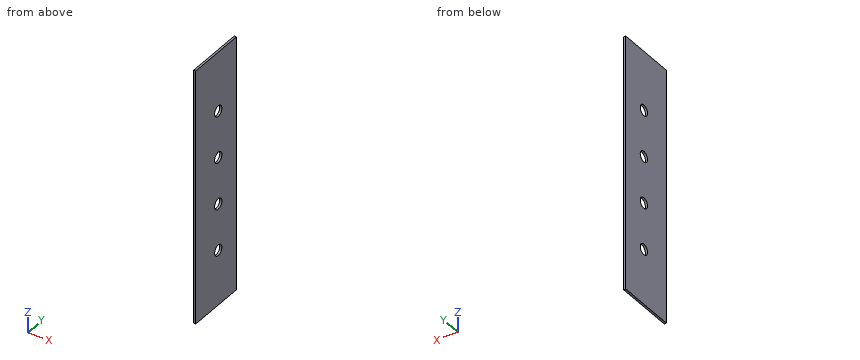
from build123d import *

# Parameters (mm, degrees)
SKETCH1_W           = 1200
SKETCH1_H           = 280
BOSS_EXTRUDE1_DEPTH = 10
SKETCH2_R           = 25
CUT_EXTRUDE1_DEPTH  = 10
LPATTERN1_COUNT     = 4
LPATTERN1_PITCH     = 220


with BuildPart() as part:
    # Sketch1 → Boss-Extrude1 (new body)
    with BuildSketch(Plane(origin=(0, 0, 0), x_dir=(0, 0, -1), z_dir=(1, 0, 0))):
        Rectangle(SKETCH1_W, SKETCH1_H)
    extrude(amount=BOSS_EXTRUDE1_DEPTH)

    # Sketch2 → Cut-Extrude1 (cut)
    with BuildSketch(Plane(origin=(10, 0, 0), x_dir=(0, 0, -1), z_dir=(1, 0, 0))):
        with Locations((-320, 15)):
            Circle(SKETCH2_R)
    cut_extrude1 = extrude(amount=-CUT_EXTRUDE1_DEPTH, mode=Mode.SUBTRACT)

    # LPattern1: Cut-Extrude1 ×4
    with Locations(*[(0, 0, -i * LPATTERN1_PITCH) for i in range(1, LPATTERN1_COUNT)]):
        add(cut_extrude1, mode=Mode.SUBTRACT)


solid = part.part
CAD build for the part. Positions are in the model's coordinates, mm. Round coordinates to 2 decimals unless told otherwise and drop trailing zeros. Write each loop counter-clockwise with the first axis right and the second up, starting at its lowest first coordinate (ties: lowest second). Pieces come first, ordered by that corner, then holes. Notation, with made-up numbers: (58, 20) -> (80, 20) arc R21 cw to (80, 37) -> close; hole circle Ø10 at (65.5, 49.25). An arc over 180 degrees is marked (long way). Answer as a JSON object with one key per item and string values.
(1) Band-saw the part on B-B, the plane x = 7.5. List the corners of the cut face in (y, z).
Reported:
{"outline": "(-140, -600) -> (140, -600) -> (140, 600) -> (-140, 600) -> close; hole circle Ø50 at (15, -340); hole circle Ø50 at (15, -120); hole circle Ø50 at (15, 100); hole circle Ø50 at (15, 320)"}
(2) Band-saw the part on A-A, the plane z = 320. List the corners of the cut face in (x, y).
Reported:
{"outline": "(0, -140) -> (10, -140) -> (10, -10) -> (0, -10) -> close; (0, 40) -> (10, 40) -> (10, 140) -> (0, 140) -> close"}
(3) Band-saw the part on C-C, the plane y = 15. List the corners of the cut face in (x, z), then the cut area to 3 significant figures.
Reported:
{"outline": "(0, -600) -> (10, -600) -> (10, -365) -> (0, -365) -> close; (0, -315) -> (10, -315) -> (10, -145) -> (0, -145) -> close; (0, -95) -> (10, -95) -> (10, 75) -> (0, 75) -> close; (0, 125) -> (10, 125) -> (10, 295) -> (0, 295) -> close; (0, 345) -> (10, 345) -> (10, 600) -> (0, 600) -> close", "area": "10,000 mm^2"}
(4) Pin check, flat tip, straight feed: P1, Ø12, axis at y = 84.5, z = -305, coming from the -X side. Stop position of the tip, or through.
Reported:
{"P1": "stops at x = 0"}
(5) Probe probe 1 along Y at (x, z) = (3.5, -340). List the from-to ranges inside material, lowest first. Write a range as [from, to].
Reported:
{"probe 1": "y = [-140, -10], [40, 140]"}
